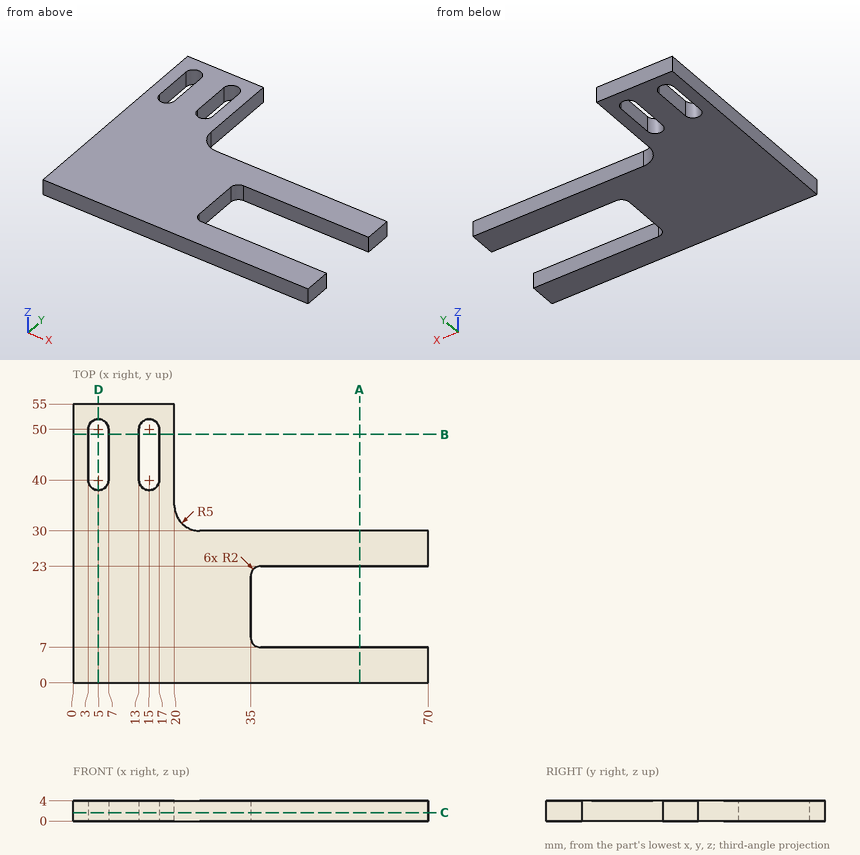
Answer from the drawing. Dimensions are ordinates in mm from the lowest x, y and z of the part. Round coordinates to 2 decimals unless told otherwise and drop trailing zeros. Loops run counter-clockwise (first coordinate to the right, second up) from the corner with the lowest first, then second, coordinate; pieces in that order, holes last. Notation, with made-up numbers: (-37.5, 49.5) - (-19.5, 49.5) arc R31 cw to (-19.5, 76.5) - close; hole circle Ø1 at (50, 7). An arc over 180 degrees is marked (long way). One line per item, written item: value.
Q1. Straight lines are drawn through the part: probe 1 along X at (y, z) = (41, 2); probe 2 along Y at (x, z) = (65.5, 0.3); probe 3 along X at (y, z) = (39.5, 2.05). For each, find the intervals that lie inside material, in ascending order.
Check values:
probe 1: 0 to 3, 7 to 13, 17 to 20
probe 2: 0 to 7, 23 to 30
probe 3: 0 to 3.06, 6.94 to 13.06, 16.94 to 20
Q2. Find section D-D on x = 5. Give the vertices of the cut face in (y, z).
Check values:
outline: (0, 0) - (38, 0) - (38, 4) - (0, 4) - close; (52, 0) - (55, 0) - (55, 4) - (52, 4) - close
Q3. Find section B-B on y = 49. Give the vertices of the cut face in (x, z).
Check values:
outline: (0, 0) - (3, 0) - (3, 4) - (0, 4) - close; (7, 0) - (13, 0) - (13, 4) - (7, 4) - close; (17, 0) - (20, 0) - (20, 4) - (17, 4) - close
Q4. Each of these flat-tipped pins is pushed along its axis until it touches: pin 1 Ø1.2 at (y, z) = (42, 1) entering from +X; pin 2 Ø2 at (y, z) = (15, 2) entering from +X; pin 3 Ø5 at (x, y) = (7, 41.5) entering from -Z. Where does it stop, or does it pass through?
Check values:
pin 1: x = 20
pin 2: x = 35
pin 3: z = 0
Q5. Find section A-A on x = 56.5. Give the vertices of the cut face in (y, z), and give its area (3 significant figures).
Check values:
outline: (0, 0) - (7, 0) - (7, 4) - (0, 4) - close; (23, 0) - (30, 0) - (30, 4) - (23, 4) - close
area: 56.0 mm2
Q6. Find section C-C on z = 1.7. Give the vertices of the cut face in (x, y).
Check values:
outline: (0, 0) - (70, 0) - (70, 7) - (37, 7) arc R2 cw to (35, 9) - (35, 21) arc R2 cw to (37, 23) - (70, 23) - (70, 30) - (25, 30) arc R5 cw to (20, 35) - (20, 55) - (0, 55) - close; hole (3, 40) arc R2 ccw to (7, 40) - (7, 50) arc R2 ccw to (3, 50) - close; hole (13, 40) arc R2 ccw to (17, 40) - (17, 50) arc R2 ccw to (13, 50) - close
